Design review of the part built by this model. Coordinates are the model's own, in mm. Coordinates: 2 decimals unless noted, no trailing zeros. Write each loop counter-clockwise with the first axis right and the second up, starting at its lowest first coordinate (ties: lowest second). Pieces come first, ordered by that corner, then holes.
Q1. Add section B-B, the plane y = 672.5. Give the boundary of the cut face in (x, z).
Q2. Clearance check with flat-ended pins moving along their axes: pin 1 Ø6 at (y, z) = (-376.5, 12) entering from -X; pin 2 Ø8 at (y, z) = (-648, 11) entering from +X; pin 3 Ø8 at (y, z) = (-346, 6) entering from -X. State where each tip first meets the part, or that it passes through.
Q3. To check wall thickness, follow probe 1 along X at (y, z) = (-277.5, 9.25); probe 2 along Y at (x, z) = (-480, 6); probe 3 along Y at (x, z) = (-482, 1.25). State the ranges of each line that lie inside material, in increasing order.
Q4. Add section A-A, the plane z = 6. Give the number of separate pieces and of enclosed holes in the cut face, plus the area to 3 significant figures.
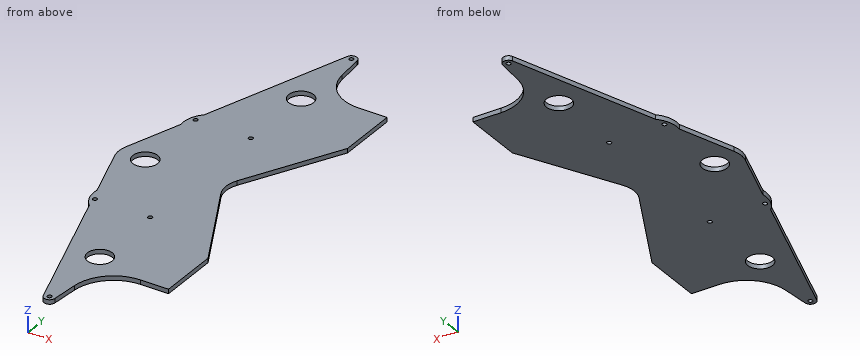
from build123d import *

# Parameters (mm, degrees)
SKETCH1_R           = 45
SKETCH1_R_2         = 3.5
SKETCH1_R_3         = 8
BOSS_EXTRUDE1_DEPTH = 16
BOSS_EXTRUDE2_START = -16
SKETCH4_R           = 3.5
BOSS_EXTRUDE2_DEPTH = 16


with BuildPart() as part:
    # Sketch1 → Boss-Extrude1 (new body)
    with BuildSketch(Plane.XY):
        with BuildLine():
            Line((-570.535490362, 31.513955821), (-503.404469767, 233.679569935))
            ThreePointArc((-503.404469767, 233.679569935), (-499.566128801, 281), (-474.336723785, 321.217323201))
            Line((-474.336723785, 321.217323201), (-298.980906816, 849.302791164))
            ThreePointArc((-298.980906816, 849.302791164), (-277.671917484, 862.864038658), (-260.076106038, 844.743114855))
            Line((-260.076106038, 844.743114855), (-251.518273259, 746.926638588))
            ThreePointArc((-251.518273259, 746.926638588), (-203.427599687, 649.408399478), (-102.089068545, 610))
            Line((-102.089068545, 610), (0, 610))
            Line((0, 610), (0, 390))
            Line((0, 390), (-176.599146277, 45.63166476))
            ThreePointArc((-176.599146277, 45.63166476), (-187.617399996, 0), (-176.599146277, -45.63166476))
            Line((-176.599146277, -45.63166476), (0, -390))
            Line((0, -390), (0, -610))
            Line((0, -610), (-102.089068545, -610))
            ThreePointArc((-102.089068545, -610), (-203.427599687, -649.408399478), (-251.518273259, -746.926638588))
            Line((-251.518273259, -746.926638588), (-260.076106038, -844.743114855))
            ThreePointArc((-260.076106038, -844.743114855), (-277.671917484, -862.864038658), (-298.980906816, -849.302791164))
            Line((-298.980906816, -849.302791164), (-474.336723785, -321.217323201))
            ThreePointArc((-474.336723785, -321.217323201), (-499.566128801, -281), (-503.404469767, -233.679569935))
            Line((-503.404469767, -233.679569935), (-570.535490362, -31.513955821))
            ThreePointArc((-570.535490362, -31.513955821), (-575.630956285, 0), (-570.535490362, 31.513955821))
        make_face()
        with Locations((-280, 562)):
            Circle(SKETCH1_R, mode=Mode.SUBTRACT)
        with Locations((-355, 582)):
            Circle(SKETCH1_R_2, mode=Mode.SUBTRACT)
        with Locations((-280, 281)):
            Circle(SKETCH1_R_3, mode=Mode.SUBTRACT)
        with Locations((-355, -582)):
            Circle(SKETCH1_R_2, mode=Mode.SUBTRACT)
        with Locations((-355, -542)):
            Circle(SKETCH1_R_2, mode=Mode.SUBTRACT)
        with Locations((-405, -20)):
            Circle(SKETCH1_R_2, mode=Mode.SUBTRACT)
        with Locations((-405, 20)):
            Circle(SKETCH1_R_2, mode=Mode.SUBTRACT)
        with Locations((-280, 843)):
            Circle(SKETCH1_R_3, mode=Mode.SUBTRACT)
        with Locations((-280, -843)):
            Circle(SKETCH1_R_3, mode=Mode.SUBTRACT)
        with Locations((-280, -281)):
            Circle(SKETCH1_R_3, mode=Mode.SUBTRACT)
        with Locations((-480, -281)):
            Circle(SKETCH1_R_3, mode=Mode.SUBTRACT)
        with Locations((-280, -562)):
            Circle(SKETCH1_R, mode=Mode.SUBTRACT)
        with Locations((-480, 0)):
            Circle(SKETCH1_R, mode=Mode.SUBTRACT)
        with Locations((-480, 281)):
            Circle(SKETCH1_R_3, mode=Mode.SUBTRACT)
        with Locations((-355, 542)):
            Circle(SKETCH1_R_2, mode=Mode.SUBTRACT)
    extrude(amount=BOSS_EXTRUDE1_DEPTH)

    # Sketch4 → Boss-Extrude2 (add)
    with BuildSketch(Plane.XY.offset(16).offset(BOSS_EXTRUDE2_START)):
        with Locations((-355, -542)):
            Circle(SKETCH4_R)
        with Locations((-355, -582)):
            Circle(SKETCH4_R)
        with Locations((-405, -20)):
            Circle(SKETCH4_R)
        with Locations((-405, 20)):
            Circle(SKETCH4_R)
        with Locations((-355, 542)):
            Circle(SKETCH4_R)
        with Locations((-355, 582)):
            Circle(SKETCH4_R)
    extrude(amount=BOSS_EXTRUDE2_DEPTH)


solid = part.part
Here are the results:
1. outline: (-357.69, 0) - (-223.92, 0) - (-223.92, 16) - (-357.69, 16) - close
2. pin 1: stops at x = -456.98
2. pin 2: stops at x = -197.19
2. pin 3: stops at x = -467.44
3. probe 1: x = -500.66 to -487.19, -472.81 to -287.19, -272.81 to -57.69
3. probe 2: y = -315.24 to -289, -273 to -45, 45 to 273, 289 to 315.24
3. probe 3: y = -312.88 to -288.75, -273.25 to -44.96, 44.96 to 273.25, 288.75 to 312.88
4. separate pieces: 1
4. enclosed holes: 9
4. area: 540,000 mm2
